Verification items for the finished model (mm, model axes). A direction names the side the tool comes from. Coordinates: 2 decimals unless noted, no trailing zeros. Loops run counter-clockwise (first coordinate to the right, second up) from the corner with the lowest first, then second, coordinate; pieces in that order, holes last.
Q1. Sectioned sample at B-B (z = -258). Enter the section's corners in (x, y).
Q2. Sectioned sample at A-A (x = -6). Enter the section's corners in (y, z), then the cut area to 3 significant figures.
Q3. Mould release check, pull along Y, two halves, no side actions. Record for faces 1 (the face through (0, -25, 7)), 2 (the face through (0, -22, 7)), 3 (the face through (-25, 0, 7)): +Y half, -Y half, draft (parallel to the pull), parting line (faces both ways), or undercut.
Q4. Material ranges on probe 1 along Y at (x, z) = (10, 415); probe 2 along X at (y, z) = (-20, 421), recorded low to high.
Q5. Access from +Z, -Z, +X, -X, +Y, -Y to the whole of each face (thin tool, end or side, straight path). Record for faces 4 (the face through (25, 0, 7)), 5 (the face through (0, 22, 7)).
```python
from build123d import *

# Parameters (mm, degrees)
GB_6728_1986_050_X_50_X_3_1_DEPTH = 1000


with BuildPart() as part:
    # Sketch1 → Gb／6728-1986方形空心型钢 050 X 50 X 3(1) (new body)
    with BuildSketch(Plane.YX.offset(-500)):
        with BuildLine():
            Line((-19, -25), (19, -25))
            ThreePointArc((19, -25), (23.242640687, -23.242640687), (25, -19))
            Line((25, -19), (25, 19))
            ThreePointArc((25, 19), (23.242640687, 23.242640687), (19, 25))
            Line((19, 25), (-19, 25))
            ThreePointArc((-19, 25), (-23.242640687, 23.242640687), (-25, 19))
            Line((-25, 19), (-25, -19))
            ThreePointArc((-25, -19), (-23.242640687, -23.242640687), (-19, -25))
        make_face()
        with BuildLine():
            Line((-19, -22), (19, -22))
            ThreePointArc((19, -22), (21.121320344, -21.121320344), (22, -19))
            Line((22, -19), (22, 19))
            ThreePointArc((22, 19), (21.121320344, 21.121320344), (19, 22))
            Line((19, 22), (-19, 22))
            ThreePointArc((-19, 22), (-21.121320344, 21.121320344), (-22, 19))
            Line((-22, 19), (-22, -19))
            ThreePointArc((-22, -19), (-21.121320344, -21.121320344), (-19, -22))
        make_face(mode=Mode.SUBTRACT)
    extrude(amount=GB_6728_1986_050_X_50_X_3_1_DEPTH)


solid = part.part
```
Geometry check:
1. outline: (-25, -19) arc R6 ccw to (-19, -25) - (19, -25) arc R6 ccw to (25, -19) - (25, 19) arc R6 ccw to (19, 25) - (-19, 25) arc R6 ccw to (-25, 19) - close; hole (-22, -19) arc R3 ccw to (-19, -22) - (19, -22) arc R3 ccw to (22, -19) - (22, 19) arc R3 ccw to (19, 22) - (-19, 22) arc R3 ccw to (-22, 19) - close
2. outline: (-25, -500) - (-22, -500) - (-22, 500) - (-25, 500) - close; (22, -500) - (25, -500) - (25, 500) - (22, 500) - close
2. area: 6,000 mm2
3. face 1: -Y half
3. face 2: undercut
3. face 3: draft
4. probe 1: y = -25 to -22, 22 to 25
4. probe 2: x = -24.92 to -21.83, 21.83 to 24.92
5. face 4: +Z, -Z, +X, +Y, -Y
5. face 5: +Z, -Z
